Input: dimensioned drawing with shaded views. Units: mm. Origin: part minimum x, y, z. Round coordinates to 2 decimals unless told otherwise and drop trailing zeros. Loops run counter-clockwise (first coordinate to the right, second up) from the corner with the lowest first, then second, coordinate; pieces in that order, holes last. Notation, with made-up numbers: M 8.25,22.5 L 60.25,22.5 A20 cw 60.25,34.5 Z; hole C -2,45 d9. An arc over 180 degrees is marked long. Return JSON: item names as keys, results as strings.
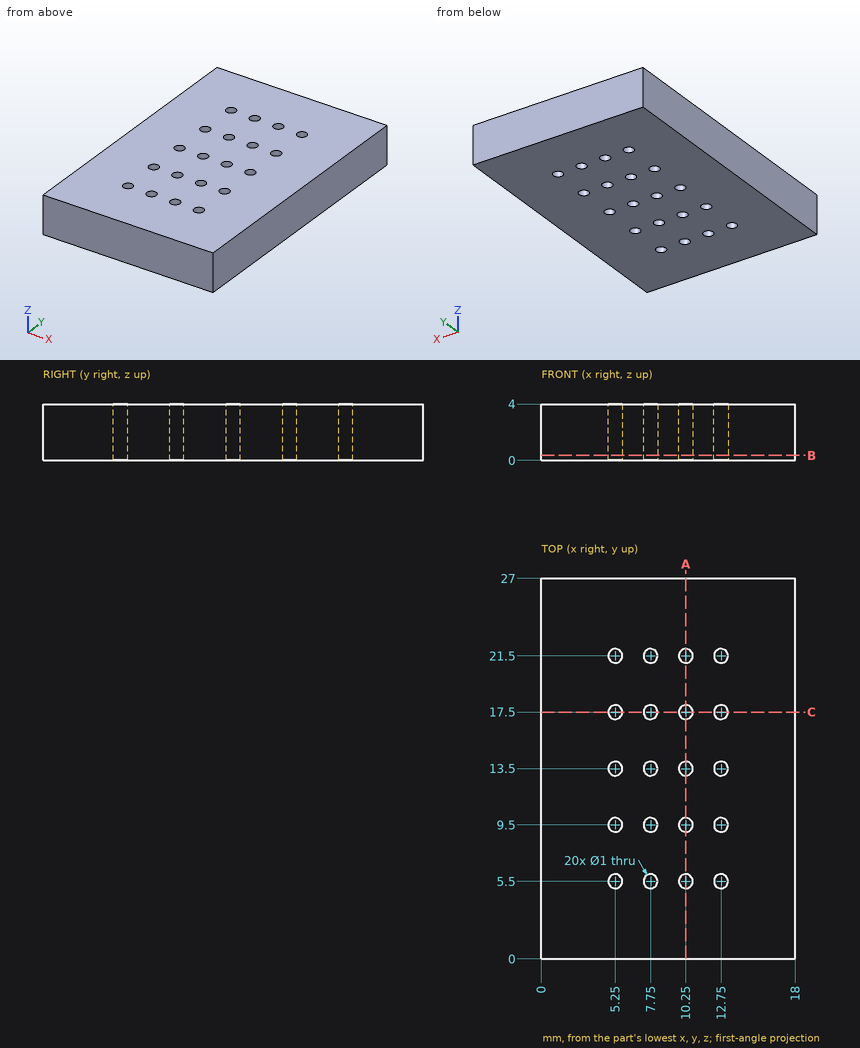
Q1. Material intervals for L1, parallel to Y at x = 7.75, z = 2.6; L2, parallel to X at y = 17.5, z = 1.6; L3, parallel to Y at x = 5, z = 2.8, sorted ascending.
Determined:
{"L1": "y = 0 to 5, 6 to 9, 10 to 13, 14 to 17, 18 to 21, 22 to 27", "L2": "x = 0 to 4.75, 5.75 to 7.25, 8.25 to 9.75, 10.75 to 12.25, 13.25 to 18", "L3": "y = 0 to 5.07, 5.93 to 9.07, 9.93 to 13.07, 13.93 to 17.07, 17.93 to 21.07, 21.93 to 27"}
Q2. Section query A-A (x = 10.25). Output: boundary loops of the cut face in (y, z), plus the area to 3 significant figures.
Determined:
{"outline": "M 0,0 L 5,0 L 5,4 L 0,4 Z; M 6,0 L 9,0 L 9,4 L 6,4 Z; M 10,0 L 13,0 L 13,4 L 10,4 Z; M 14,0 L 17,0 L 17,4 L 14,4 Z; M 18,0 L 21,0 L 21,4 L 18,4 Z; M 22,0 L 27,0 L 27,4 L 22,4 Z", "area": "88.0 mm^2"}
Q3. Section query B-B (z = 0.35). State how many separate pieces and enclosed holes the cut face has, plus the area to 3 significant figures.
Determined:
{"separate pieces": "1", "enclosed holes": "20", "area": "470 mm^2"}
Q4. Section query C-C (y = 17.5). Output: boundary loops of the cut face in (x, z), plus the area to 3 significant figures.
Determined:
{"outline": "M 0,0 L 4.75,0 L 4.75,4 L 0,4 Z; M 5.75,0 L 7.25,0 L 7.25,4 L 5.75,4 Z; M 8.25,0 L 9.75,0 L 9.75,4 L 8.25,4 Z; M 10.75,0 L 12.25,0 L 12.25,4 L 10.75,4 Z; M 13.25,0 L 18,0 L 18,4 L 13.25,4 Z", "area": "56.0 mm^2"}
